The model under review builds one solid part; all positions refer to its coordinate system, in mm. A direction names the side the tool comes from. Round coordinates to 2 decimals unless told otherwise and drop trailing zeros. Write each loop counter-clockwise with the first axis right and the second up, starting at its lowest first coordinate (ties: lowest second). Pieces come first, ordered by that corner, then holes. Notation, with made-up numbers: (45, 2.5) -> (99, 2.5) arc R30 ccw to (99, 36.5) -> close; hole circle Ø6 at (17.25, -18.5). An arc over 180 degrees is marked (long way). Use CSV: the item, a comma, the result in double quotes. Start each with the question number.
1) Wall thickness on probe 1 along Y at (x, z) = (99, 4.25); probe 2 along Y at (x, z) = (0, 5.5) (3 decimals); probe 3 along X at (y, z) = (5, 1.75): over which ranges is each line inside the solid? List them lowest first. Write a range as [from, to].
2) Take a section at C-C, the plane x = 95. Give the boundary of the cut face in (y, z).
3) Take a section at B-B, the plane z = 5. State how many separate pieces and enclosed holes the cut face has, then the cut area to 3 significant figures.
4) Machinability: for faces 5 (the face through (42.826, -10.099, 5.07)), 6 (the face through (13.928, -18.744, 5.07)), which of the approach directions +Z, -Z, +X, -X, +Y, -Y give a long, thin tool a straight path to every point of the face, cutting with its end or side? Answer none if there is none.
5) Take a section at A-A, the plane x = 13. Give the boundary of the cut face in (y, z).
6) Mouldability with a two-part tool opening along X and no side actions: class faces 1 (the face through (21.39, 12.26, 5.07)), 2 (the face through (47, 0, 10)), 3 (the face through (119, 0, 5)), 4 (the face through (43.294, -1.054, 4.93)) as released by +X, released by -X, zero draft, split by the parting line, or undercut.
7) For pin 1 Ø1.5 at (x, z) = (98, 4) entering from +Y; pin 2 Ø1.9 at (x, y) = (99, 13.5) entering from -Z; pin 3 Ø2 at (x, z) = (63.5, 7.5) entering from -Y; pin 4 Ø3 at (x, y) = (8, -16) entering from -Z, all flat-tipped, find the tip position at first contact; note any pin that passes through.
from build123d import *

# Parameters (mm, degrees)
SKETCH_1_R          = 14.575
SKETCH_1_R_2        = 10
EXTRUDE_1_DEPTH     = 10
CUT_EXTRUDE_START   = -10
CUT_EXTRUDE_1_DEPTH = 10
FILLET_1_R          = 4
SKETCH_3_R          = 1.6
CUT_EXTRUDE_2_DEPTH = 10
CUT_EXTRUDE_3_DEPTH = 10
FILLET_2_R          = 10


with BuildPart() as part:
    # 草图1 → 凸台-拉伸1 (new body)
    with BuildSketch(Plane.XY):
        with BuildLine():
            ThreePointArc((0.58717803, 22.567362428), (-22.575, 0), (0.58717803, -22.567362428))
            Line((0.58717803, -22.567362428), (99.52020202, -19.993233602))
            ThreePointArc((99.52020202, -19.993233602), (119, 0), (99.52020202, 19.993233602))
            Line((99.52020202, 19.993233602), (0.58717803, 22.567362428))
        make_face()
        Circle(SKETCH_1_R, mode=Mode.SUBTRACT)
        with Locations((99, 0)):
            Circle(SKETCH_1_R_2, mode=Mode.SUBTRACT)
    extrude(amount=EXTRUDE_1_DEPTH)

    # 草图2 → 切除-拉伸1 (cut)
    with BuildSketch(Plane.XY.offset(10).offset(CUT_EXTRUDE_START)):
        with BuildLine():
            Line((77.045246178, 12.575299839), (17.612754311, 14.121668123))
            ThreePointArc((17.612754311, 14.121668123), (21.298339766, 7.484072969), (22.575, 0))
            ThreePointArc((22.575, 0), (21.923337, -5.384971659), (20.005970563, -10.459051908))
            Line((20.005970563, -10.459051908), (77.045246178, 12.575299839))
        make_face()
        with BuildLine():
            Line((81.037736343, 8.795287621), (24.748948749, -13.935992167))
            Line((24.748948749, -13.935992167), (83.317534331, -12.412101777))
            ThreePointArc((83.317534331, -12.412101777), (79.114570809, -2.137687039), (81.037736343, 8.795287621))
        make_face()
    extrude(amount=CUT_EXTRUDE_1_DEPTH, mode=Mode.SUBTRACT)

    # 圆角1
    fillet_1_edges = [part.edges().sort_by_distance(p)[0] for p in [
        (81.037736343, 8.795287621, 5),
        (83.317534331, -12.412101777, 5),
        (24.748948749, -13.935992167, 5),
        (20.005970563, -10.459051908, 5),
        (17.612754311, 14.121668123, 5),
        (77.045246178, 12.575299839, 5),
    ]]
    fillet(fillet_1_edges, radius=FILLET_1_R)

    # 草图3 → 切除-拉伸2 (cut)
    with BuildSketch(Plane.XY.offset(10)):
        with Locations((99, 13.5)):
            Circle(SKETCH_3_R)
        with Locations((110.691342951, 6.75)):
            Circle(SKETCH_3_R)
        with Locations((110.691342951, -6.75)):
            Circle(SKETCH_3_R)
        with Locations((99, -13.5)):
            Circle(SKETCH_3_R)
        with Locations((87.308657049, -6.75)):
            Circle(SKETCH_3_R)
        with Locations((87.308657049, 6.75)):
            Circle(SKETCH_3_R)
    extrude(amount=-CUT_EXTRUDE_2_DEPTH, mode=Mode.SUBTRACT)

    # 草图4 → 切除-拉伸3 (cut)
    with BuildSketch(Plane.XY.offset(10)):
        Polygon((0.58717803, -22.567362428), (31.302336493, -13.765480202), (40.58717803, -21.526606279), align=None)
    extrude(amount=-CUT_EXTRUDE_3_DEPTH, mode=Mode.SUBTRACT)

    # 圆角2
    fillet_2_edges = [part.edges().sort_by_distance(p)[0] for p in [
        (0.58717803, -22.567362428, 5),
        (40.58717803, -21.526606279, 5),
        (31.302336493, -13.765480202, 5),
    ]]
    fillet(fillet_2_edges, radius=FILLET_2_R)


solid = part.part
Values found:
1,probe 1,"[-20.01, -15.1], [-11.9, -10], [10, 11.9], [15.1, 20.01]"
1,probe 2,"[-22.523, -14.575], [14.575, 22.575]"
1,probe 3,"[-22.01, -13.69], [13.69, 22.01], [58.29, 71.64], [77.82, 90.34], [107.66, 118.36]"
2,outline,"(-20.11, 0) -> (-9.17, 0) -> (-9.17, 10) -> (-20.11, 10) -> close; (9.17, 0) -> (20.11, 0) -> (20.11, 10) -> (9.17, 10) -> close"
3,separate pieces,"1"
3,enclosed holes,"10"
3,area,"3,380 mm²"
4,face 5,"+Z, -Z"
4,face 6,"+Z, -Z, -Y"
5,outline,"(-19.01, 0) -> (-6.59, 0) -> (-6.59, 10) -> (-19.01, 10) -> close; (6.59, 0) -> (22.24, 0) -> (22.24, 10) -> (6.59, 10) -> close"
6,face 1,"undercut"
6,face 2,"zero draft"
6,face 3,"released by +X"
6,face 4,"undercut"
7,pin 1,"y = 20.05"
7,pin 2,"through"
7,pin 3,"y = -20.96"
7,pin 4,"z = 0"
